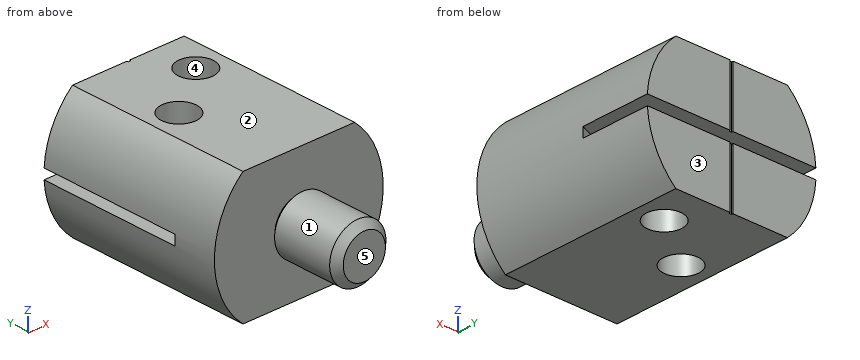
from build123d import *

# Parameters (mm, degrees)
SKETCH1_R           = 6
BOSS_EXTRUDE1_DEPTH = 18
SKETCH2_OUTSIDE_W   = 18.948
SKETCH2_OUTSIDE_H   = 18.948
SKETCH2_OUTSIDE_R   = 2
CUT_EXTRUDE1_DEPTH  = 5
CUT_EXTRUDE2_DEPTH  = 0.35
CHAMFER1_SIZE       = 0.5
SKETCH6_W           = 0.3
SKETCH6_H           = 0.3
SKETCH9_OUTSIDE_W   = 18.948
SKETCH9_OUTSIDE_H   = 18.948
SKETCH9_OUTSIDE_W_2 = 12.764596016
SKETCH9_OUTSIDE_H_2 = 9
CUT_EXTRUDE3_DEPTH  = 20.899748742
M3_TAPPED_HOLE1_D   = 2.5
SKETCH14_W          = 0.2
SKETCH14_H          = 9
CUT_EXTRUDE5_DEPTH  = 0.1


with BuildPart() as part:
    # Sketch1 → Boss-Extrude1 (new body)
    with BuildSketch(Plane(origin=(0, 0, 0), x_dir=(1, 0, 0), z_dir=(0, 1, 0))):
        with Locations(Location((0, 0, 0), (0, 0, 270))):
            Circle(SKETCH1_R)
    extrude(amount=BOSS_EXTRUDE1_DEPTH)

    # Sketch2 outside → Cut-Extrude1 (cut)
    with BuildSketch(Plane.XZ):
        Rectangle(SKETCH2_OUTSIDE_W, SKETCH2_OUTSIDE_H)
        with Locations(Location((0, 0, 0), (0, 0, 270))):
            Circle(SKETCH2_OUTSIDE_R, mode=Mode.SUBTRACT)
    extrude(amount=-CUT_EXTRUDE1_DEPTH, mode=Mode.SUBTRACT)

    # Sketch8 → Cut-Extrude2 (cut, symmetric)
    with BuildSketch(Plane.XY):
        Polygon((-6, 8), (6, 13.093697795), (6, 18), (-6, 18), align=None)
    extrude(amount=CUT_EXTRUDE2_DEPTH, both=True, mode=Mode.SUBTRACT)

    # Chamfer1
    chamfer1_edges = [part.edges().sort_by_distance(p)[0] for p in [
        (0, 0, 2),
    ]]
    chamfer(chamfer1_edges, length=CHAMFER1_SIZE)

    # Sketch6 → Cut-Revolve1 (revolve, cut)
    with BuildSketch(Plane.XY, mode=Mode.PRIVATE) as cut_revolve1_sk:
        with Locations((1.85, 4.85)):
            Rectangle(SKETCH6_W, SKETCH6_H)
    revolve(cut_revolve1_sk.sketch.rotate(Axis((0, 0, 0), (0, 1, 0)), 90), axis=Axis((0, 0, 0), (0, 1, 0)), mode=Mode.SUBTRACT)

    # Sketch9 outside → Cut-Extrude3 (cut, through all)
    with BuildSketch(Plane(origin=(0, 18, 0), x_dir=(1, 0, 0), z_dir=(0, 1, 0))):
        Rectangle(SKETCH9_OUTSIDE_W, SKETCH9_OUTSIDE_H)
        Rectangle(SKETCH9_OUTSIDE_W_2, SKETCH9_OUTSIDE_H_2, mode=Mode.SUBTRACT)
    extrude(amount=-CUT_EXTRUDE3_DEPTH, mode=Mode.SUBTRACT)

    # M3 Tapped Hole1 (through all)
    with Locations(Plane.XY.offset(4.5)):
        with Locations((2, 15), (-2, 12)):
            Hole(M3_TAPPED_HOLE1_D / 2)

    # Sketch14 → Cut-Extrude5 (cut)
    with BuildSketch(Plane(origin=(0, 18, 0), x_dir=(1, 0, 0), z_dir=(0, 1, 0))):
        Rectangle(SKETCH14_W, SKETCH14_H)
    extrude(amount=-CUT_EXTRUDE5_DEPTH, mode=Mode.SUBTRACT)


solid = part.part
Source: CAD feature listing. Evaluate the final solid. Frame: model axes, mm. Face numbers are marked on the shaded views. A direction names the side the tool comes from. Round coordinates to 2 decimals unless told otherwise and drop trailing zeros. Loops run counter-clockwise (first coordinate to the right, second up) from the corner with the lowest first, then second, coordinate; pieces in that order, holes last. Notation, with made-up numbers: (3.5, 4) - (48.5, 4) arc R28 ccw to (48.5, 26) - close; hole circle Ø6 at (64, 89.25). An arc over 180 degrees is marked (long way). Write item = value, one per line. Start each with the question number.
(1) Section query A-A, the plane y = 15. Output: boundary loops of the cut face in (x, z), plus the area to 3 significant figures.
(2) Set-up query: the marked faces 1 and 2. Return all of +Z, -Z, +X, -X, +Y, -Y with unobstructed straight access to the full face (end or side cutting, diameter ignored); none if empty.
(3) Section query D-D, the plane y = 12. Output: boundary loops of the cut face in (x, z).
(4) Section query B-B, the plane z = 0. Output: boundary loops of the cut face in (x, y).
(5) Ray query, line 1 along Y through (x, z) = (2, -1.55); line 2 along Z through (x, y) = (0.75, 15.75); line 3 along Y through (x, z) = (-2, -1.25). Return the intervals inside material, ascending. Write a range as from..to.
(6) Pull-direction query (Y, two-part tool) for the marked faces 3, 4 and 5; classes: +Y half, -Y half, draft (parallel to the pull), parting line (faces both ways), or undercut.
(7) Pin query (flat end, axial travel): pin 1 (1.5 mm diameter, centred on x = 4.5, z = 2.5, fed in from -Y); pin 2 (2 mm diameter, centred on x = 2, y = 15, fed in from -Z); pin 3 (1 mm diameter, centred on y = 2.5, z = -1, fed in from -X). Return the tip coordinate at first contact, or that it passes through.
(8) Section query C-C, the plane x = 2.25. Output: boundary loops of the cut face in (y, z), plus the area to 3 significant figures.
Conclusion:
q1.outline = (-5.99, -0.35) arc R6 ccw to (-3.97, -4.5) - (0.75, -4.5) - (0.75, -0.35) - close; (-5.99, 0.35) - (0.75, 0.35) - (0.75, 4.5) - (-3.97, 4.5) arc R6 ccw to start; (3.25, -4.5) - (3.97, -4.5) arc R6 ccw to (5.99, -0.35) - (3.25, -0.35) - close; (3.25, 0.35) - (5.99, 0.35) arc R6 ccw to (3.97, 4.5) - (3.25, 4.5) - close
q1.area = 67.6 mm2
q2.face_1 = -Y
q2.face_2 = +Z, +X, -X, +Y, -Y
q3.outline = (-5.99, -0.35) arc R6 ccw to (-3.97, -4.5) - (-3.25, -4.5) - (-3.25, -0.35) - close; (-5.99, 0.35) - (-3.25, 0.35) - (-3.25, 4.5) - (-3.97, 4.5) arc R6 ccw to start; (-0.75, -4.5) - (3.97, -4.5) arc R6 ccw to (3.97, 4.5) - (-0.75, 4.5) - (-0.75, 0.35) - (3.42, 0.35) - (3.42, -0.35) - (-0.75, -0.35) - close
q4.outline = (-6, 5) - (-1.7, 5) - (-1.7, 4.7) - (-2, 4.7) - (-2, 0.5) - (-1.5, 0) - (1.5, 0) - (2, 0.5) - (2, 4.7) - (1.7, 4.7) - (1.7, 5) - (6, 5) - (6, 13.09) - (-6, 8) - close
q5.line_1 = 5..13.75, 16.25..18
q5.line_2 = -4.5..-0.35, 0.35..4.5
q5.line_3 = 5..10.75, 13.25..18
q6.face_3 = +Y half
q6.face_4 = undercut
q6.face_5 = -Y half
q7.pin_1 = 5
q7.pin_2 = through
q7.pin_3 = -1.94
q8.outline = (5, -4.5) - (13.78, -4.5) - (13.78, -0.35) - (11.5, -0.35) - (11.5, 0.35) - (13.78, 0.35) - (13.78, 4.5) - (5, 4.5) - close; (16.22, -4.5) - (18, -4.5) - (18, -0.35) - (16.22, -0.35) - close; (16.22, 0.35) - (18, 0.35) - (18, 4.5) - (16.22, 4.5) - close
q8.area = 92.1 mm2
